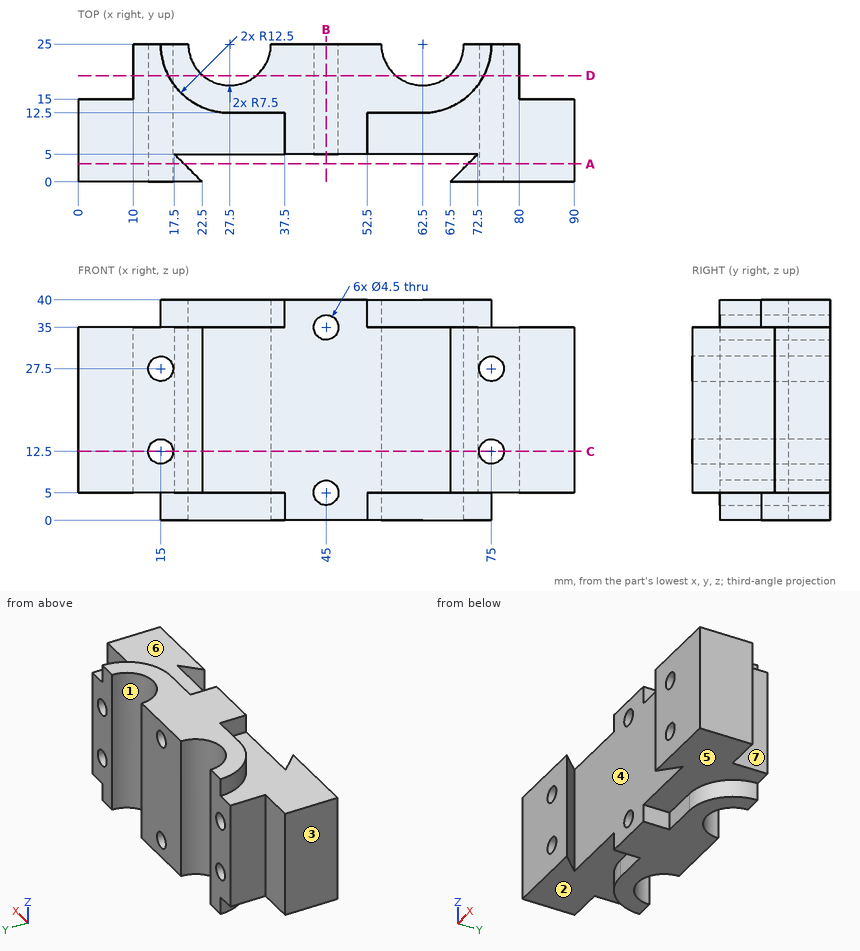
Check sheet for the drawn part. Datum: minimum x, y, z corner. Units: mm. A direction names the side the tool comes from. Coordinates: 2 decimals unless noted, no trailing zeros. Loops run counter-clockwise (first coordinate to the right, second up) from the corner with the lowest first, then second, coordinate; pieces in that order, holes last. Notation, with made-up numbers: (70, -28) -> (101, -28) arc R12 cw to (101, -13) -> close; hole circle Ø2 at (67.25, -37.5). An arc over 180 degrees is marked (long way). Answer as CSV lines item,"result".
1) Cross-section at B-B, the plane x = 45. Record the cut outline in (y, z).
Found:
outline,"(5, 0) -> (25, 0) -> (25, 2.75) -> (5, 2.75) -> close; (5, 7.25) -> (25, 7.25) -> (25, 32.75) -> (5, 32.75) -> close; (5, 37.25) -> (25, 37.25) -> (25, 40) -> (5, 40) -> close"
2) Depth check by flat-ended pin: pin 1 (4 mm diameter, centred on x = 34.5, z = 37.5, fed in from -Y); pin 2 (5 mm diameter, centred on x = 85.5, z = 26.5, fed in from +Y); pin 3 (3 mm diameter, centred on y = 18, z = 29, fed in from -X). Enter the tip coordinate at first touch or a pass-through.
Found:
pin 1,"stops at y = 12.5"
pin 2,"stops at y = 15"
pin 3,"stops at x = 10"
3) Tool access check on the marked faces 5, 6 and 7. Record the directions out of +Z, -Z, +X, -X, +Y, -Y that give a thin tool (end or side, any length) a straight path to the whole face; none if there is none.
Found:
face 5,"-Z, +X, -Y"
face 6,"+Z, +X, -Y"
face 7,"+Z, -Z, +X, +Y"
4) Cross-section at C-C, the plane z = 12.5. Record the cut outline in (x, y).
Found:
outline,"(0, 0) -> (12.75, 0) -> (12.75, 25) -> (10, 25) -> (10, 15) -> (0, 15) -> close; (17.25, 0) -> (22.5, 0) -> (17.5, 5) -> (72.5, 5) -> (67.5, 0) -> (72.75, 0) -> (72.75, 25) -> (70, 25) arc R7.5 cw to (55, 25) -> (35, 25) arc R7.5 cw to (20, 25) -> (17.25, 25) -> close; (77.25, 0) -> (90, 0) -> (90, 15) -> (80, 15) -> (80, 25) -> (77.25, 25) -> close"
5) Thickness scan on L1, parallel to Z at x = 75, y = 18.75; L2, parallel to X at y = 23, z = 27; L3, parallel to X at y = 23.5, z = 14.5. Record the ranges inside material, lowest first. Write a range as from..to.
Found:
L1,"z = 5..10.25, 14.75..25.25, 29.75..35"
L2,"x = 10..12.81, 17.19..20.27, 34.73..55.27, 69.73..72.81, 77.19..80"
L3,"x = 10..13.97, 16.03..20.15, 34.85..55.15, 69.85..73.97, 76.03..80"
6) Release check for a two-part mould opening along X. For the marked faces 1, 2, 3 and 4 record: +X half, -X half, draft (parallel to the pull), parting line (faces both ways), or undercut.
Found:
face 1,"undercut"
face 2,"draft"
face 3,"-X half"
face 4,"undercut"
7) Cross-section at A-A, the plane y = 3.25. Record the cut outline in (x, z).
Found:
outline,"(0, 5) -> (19.25, 5) -> (19.25, 35) -> (0, 35) -> close; (70.75, 5) -> (90, 5) -> (90, 35) -> (70.75, 35) -> close; hole circle Ø4.5 at (15, 12.5); hole circle Ø4.5 at (15, 27.5); hole circle Ø4.5 at (75, 12.5); hole circle Ø4.5 at (75, 27.5)"
8) Cross-section at D-D, the plane y = 19.25. Count the separate pieces of the cut face and the enclosed holes in it, then the cut area to 3 significant figures.
Found:
separate pieces,"3"
enclosed holes,"6"
area,"1,810 mm2"
